Check sheet for the drawn part. Datum: minimum x, y, z corner. Units: mm. Round coordinates to 2 decimals unless told otherwise and drop trailing zeros. Write each loop counter-clockwise with the first axis right and the second up, starting at its lowest first coordinate (ties: lowest second). Pieces come first, ordered by that corner, then holes. Notation, with made-up numbers: M 22.5,-20.5 L 32.5,-20.5 A33 ccw 32.5,10.5 Z; hole C -26,59.5 d6. An arc over 180 degrees is marked long. Use a Markdown table: item, result.
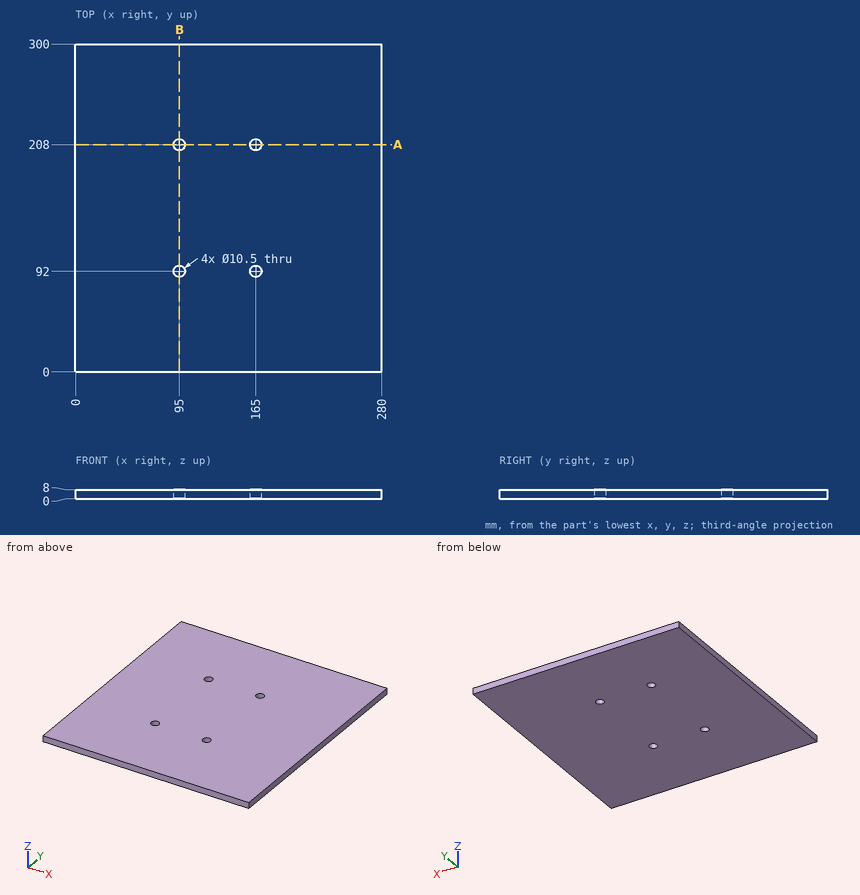
Item 1: Material ranges on line 1 along X through (y, z) = (208, 1.5); line 2 along Y through (x, z) = (165, 5.75), recorded low to high. Write a range as from..to.
Outcome:
| item | result |
|---|---|
| line 1 | x = 0..89.75, 100.25..159.75, 170.25..280 |
| line 2 | y = 0..86.75, 97.25..202.75, 213.25..300 |
Item 2: Cross-section at B-B, the plane x = 95. Record the cut outline in (y, z).
Outcome:
| item | result |
|---|---|
| outline | M 0,0 L 86.75,0 L 86.75,8 L 0,8 Z; M 97.25,0 L 202.75,0 L 202.75,8 L 97.25,8 Z; M 213.25,0 L 300,0 L 300,8 L 213.25,8 Z |
Item 3: Go/stop test with flat-tipped pins: pin 1 (1.5 mm diameter, centred on x = 67, y = 62.5, fed in from -Z); pin 2 (8.5 mm diameter, centred on x = 95, y = 208, fed in from +Z) (1 decimal). Record where each tip stops, or that it passes through.
Outcome:
| item | result |
|---|---|
| pin 1 | stops at z = 0 |
| pin 2 | passes through |
Item 4: Cross-section at A-A, the plane y = 208. Record the cut outline in (x, z), and give its area (3 significant figures).
Outcome:
| item | result |
|---|---|
| outline | M 0,0 L 89.75,0 L 89.75,8 L 0,8 Z; M 100.25,0 L 159.75,0 L 159.75,8 L 100.25,8 Z; M 170.25,0 L 280,0 L 280,8 L 170.25,8 Z |
| area | 2,070 mm2 |
